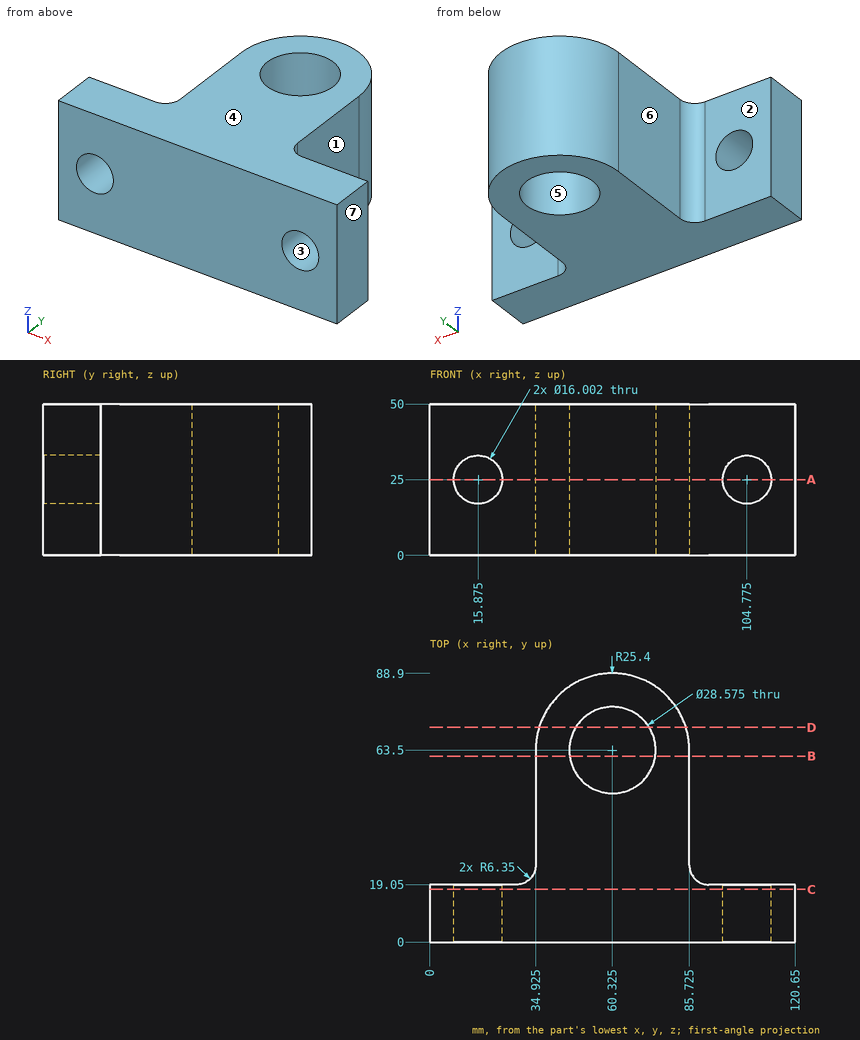
Study the drawing (mm; zero at the part's minimum x, y, z) and answer. A direction names the side the tool comes from. Round coordinates to 2 decimals unless told otherwise and drop trailing zeros. Loops run counter-clockwise (first coordinate to the right, second up) from the corner with the lowest first, then second, coordinate; pieces in that order, holes last.
Q1. Section A-A, the plane z = 25 is taken. Count the separate pieces of the cut face and the enclosed holes in it, then the cut area to 3 significant figures.
Q2. Section B-B, the plane y = 61.5 is taken. Determine the outline of the cut face in (x, z) (3 decimals), then the cut area to 3 significant figures.
Q3. Which of the six approach directions +Z, -Z, +X, -X, +Y, -Y give full straight-line access (tool end or side, diameter ignored) to the marked faces 1, 2 and 3?
Q4. Section C-C, the plane y = 17.5 is taken. Determine the outline of the cut face in (x, z) (3 decimals).
Q5. Find the intervals of material crossed by line 1 (X direction, y = 8, z = 25); line 2 (X direction, y = 63, z = 33) (3 decimals); line 3 (X direction, y = 12, z = 19), in increasing order.
Q6. Section D-D, the plane y = 71 is taken. Determine the outline of the cut face in (x, z), then the cut area to 3 significant figures.
Q7. Given pin 1 Ø12 at (x, z) = (88, 5.5) entering from -Y; pin 2 Ø1.5 at (y, z) = (79.5, 44) entering from -X; pin 3 Ø1 at (x, z) = (72.5, 13) entering from +Y; pin 4 Ø1 at (x, z) = (21.5, 44) entering from +Y, each flat-ended and moving along its own axis, determine where each tip first touches the part or whether it passes through.
Q8. For a pull along X with two mould halves and no side action, classify the marked faces 4, 5, 6 and 7 as released by +X, released by -X, zero draft, split by the parting line, or undercut.
Completed:
1. separate pieces: 3
1. enclosed holes: 1
1. area: 4,340 mm2
2. outline: (34.925, 0) - (46.178, 0) - (46.178, 50) - (34.925, 50) - close; (74.472, 0) - (85.725, 0) - (85.725, 50) - (74.472, 50) - close
2. area: 1,130 mm2
3. face 1: +Z, -Z, +X, +Y
3. face 2: +Z, -Z, -X, +Y
3. face 3: +Y, -Y
4. outline: (0, 0) - (120.65, 0) - (120.65, 50) - (0, 50) - close; hole circle Ø16.002 at (15.875, 25); hole circle Ø16.002 at (104.775, 25)
5. line 1: x = 0 to 7.87, 23.88 to 96.77, 112.78 to 120.65
5. line 2: x = 34.925 to 46.046, 74.604 to 85.725
5. line 3: x = 0 to 10.58, 21.17 to 99.48, 110.07 to 120.65
6. outline: (36.06, 0) - (48.16, 0) - (48.16, 50) - (36.06, 50) - close; (72.49, 0) - (84.59, 0) - (84.59, 50) - (72.49, 50) - close
6. area: 1,210 mm2
7. pin 1: stops at y = 0
7. pin 2: stops at x = 40.01
7. pin 3: stops at y = 86.06
7. pin 4: stops at y = 19.05
8. face 4: zero draft
8. face 5: undercut
8. face 6: released by -X
8. face 7: released by +X
